```python
from build123d import *

# Parameters (mm, degrees)
BRACKET_SIDE_PROFILE_SKETCH_R        = 3
BRACKET_BODY_EXTRUDE_70MM_DEPTH      = 35
OUTLINE_AND_KEYHOLE_CUT_DEPTH        = 89.24823725
OUTLINE_AND_KEYHOLE_CUT_DEPTH_BACK   = 89.24823725
OUTLINE_AND_KEYHOLE_SKETCH_OUTSIDE_W = 94.54
OUTLINE_AND_KEYHOLE_SKETCH_OUTSIDE_H = 110.471


with BuildPart() as part:
    # Bracket Side Profile Sketch → Bracket Body Extrude 70mm (new, symmetric)
    with BuildSketch(Plane(origin=(0, 0, 0), x_dir=(0, 0, -1), z_dir=(1, 0, 0))):
        with BuildLine():
            Line((1.25, 5.868347297), (1.25, 38))
            ThreePointArc((1.25, 38), (-1.509366946, 51.872274423), (-9.367379182, 63.632620818))
            ThreePointArc((-9.367379182, 63.632620818), (-11.930194847, 69.819805153), (-9.367379182, 76.006989489))
            ThreePointArc((-9.367379182, 76.006989489), (-8.164290412, 77.807539075), (-7.741821818, 79.931432124))
            Line((-7.741821818, 79.931432124), (-10.241821818, 79.931432124))
            ThreePointArc((-10.241821818, 79.931432124), (-10.473989243, 78.764247656), (-11.135146135, 77.774756442))
            ThreePointArc((-11.135146135, 77.774756442), (-14.430194847, 69.819805153), (-11.135146135, 61.864853865))
            ThreePointArc((-11.135146135, 61.864853865), (-3.819065778, 50.915565842), (-1.25, 38))
            Line((-1.25, 38), (-1.25, 5.868347297))
            ThreePointArc((-1.25, 5.868347297), (0, -6), (1.25, 5.868347297))
        make_face()
        Circle(BRACKET_SIDE_PROFILE_SKETCH_R, mode=Mode.SUBTRACT)
    extrude(amount=BRACKET_BODY_EXTRUDE_70MM_DEPTH, both=True)

    # Outline and Keyhole Sketch outside → Outline and Keyhole Cut (cut, two sides: drawn at the far end of the back side and taken through both)
    # profile 1 of 2: a face of its own
    with BuildSketch(Plane.XY.offset(1.25).offset(-OUTLINE_AND_KEYHOLE_CUT_DEPTH_BACK)):
        with Locations((0, 36.9655)):
            Rectangle(OUTLINE_AND_KEYHOLE_SKETCH_OUTSIDE_W, OUTLINE_AND_KEYHOLE_SKETCH_OUTSIDE_H)
        with BuildLine():
            Line((35, -6), (35, 17))
            ThreePointArc((35, 17), (33.314760402, 27.729712921), (28.421329179, 37.426160865))
            ThreePointArc((28.421329179, 37.426160865), (22.418139751, 49.027821234), (20, 61.864853865))
            Line((20, 61.864853865), (20, 79.931432124))
            Line((20, 79.931432124), (-20, 79.931432124))
            Line((-20, 79.931432124), (-20, 61.864853865))
            ThreePointArc((-20, 61.864853865), (-22.418139751, 49.027821234), (-28.421329179, 37.426160865))
            ThreePointArc((-28.421329179, 37.426160865), (-33.314760402, 27.729712921), (-35, 17))
            Line((-35, 17), (-35, -6))
            Line((-35, -6), (-15, -6))
            Line((-15, -6), (-15, 9))
            Line((-15, 9), (15, 9))
            Line((15, 9), (15, -6))
            Line((15, -6), (35, -6))
        make_face(mode=Mode.SUBTRACT)
    # profile 2 of 2: a face of its own
    with BuildSketch(Plane.XY.offset(1.25).offset(-OUTLINE_AND_KEYHOLE_CUT_DEPTH_BACK)):
        with BuildLine():
            Line((7, 49), (7, 39.124143795))
            ThreePointArc((7, 39.124143795), (0, 18.5), (-7, 39.124143795))
            Line((-7, 39.124143795), (-7, 49))
            ThreePointArc((-7, 49), (0, 56), (7, 49))
        make_face()
    extrude(amount=OUTLINE_AND_KEYHOLE_CUT_DEPTH + OUTLINE_AND_KEYHOLE_CUT_DEPTH_BACK, mode=Mode.SUBTRACT)


solid = part.part
```
Input: part model. Units: mm. Frame: model coordinates. A direction names the side the tool comes from. Round coordinates to 2 decimals unless told otherwise and drop trailing zeros. Loops run counter-clockwise (first coordinate to the right, second up) from the corner with the lowest first, then second, coordinate; pieces in that order, holes last. Notation, with made-up numbers: M 47,-24 L 65,-24 A22 cw 65,1 Z; hole C -13.5,5 d10. An arc over 180 degrees is marked long. Answer in a Markdown table with one row per item. Add a question column.
1. Section A-A (y = 0). Output: boundary loops of the cut face in (x, z).
2. Contact query for flat-ended pins moving along their axis: pin 1 (10 mm diameter, centred on x = 17.5, y = 15, fed in from -Z); pin 2 (1 mm diameter, centred on x = 7.5, y = 51.5, fed in from -Z); pin 3 (1.3 mm diameter, centred on y = 43.5, z = 0, fed in from -X); pin 4 (3 mm diameter, centred on x = -26.5, y = 43.5, fed in from +Z). Output: stop coordinate, or through.
3. Mould query, pull axis Z, two halves, no side actions, for faces 1 (the face through (-25, 0, 3)), 2 (the face through (25, -6, 0)), 3 (the face through (0.4, 18.507, -0.008)), 4 (the face through (0.28, 78.78, 10.468)). Classes: released by +Z, released by -Z, zero draft, split by the parting line, or undercut.
4. Section C-C (x = -9.5). Output: boundary loops of the cut face in (y, z).
5. Set-up query: faces 5 (the face through (0, 18, -1.25)), 6 (the face through (0.39, 57.31, 4.32)), 7 (the face through (-20, 71, 13)), 8 (the face through (0, 15, 1.25)). Return all of +Z, -Z, +X, -X, +Y, -Y with unobstructed straight access to the full face (end or side cutting, diameter ignored); none if empty.
6. Section D-D (y = 30). Output: boundary loops of the cut face in (x, z), and give its area (3 significant figures).
7. Section B-B (x = -17). Output: boundary loops of the cut face in (y, z), and give its area (3 significant figures).
8. Ray query, probe 1 along Z at (x, y) = (-25, 0); probe 2 along Z at (x, y) = (-15, 11); probe 3 along Y at (x, z) = (-25, 0). Return the intervals inside material, ascending.
Values follow:
| question | item | result |
|---|---|---|
| 1 | outline | M -35,-6 L -15,-6 L -15,-3 L -35,-3 Z; M -35,3 L -15,3 L -15,6 L -35,6 Z; M 15,-6 L 35,-6 L 35,-3 L 15,-3 Z; M 15,3 L 35,3 L 35,6 L 15,6 Z |
| 2 | pin 1 | z = -1.25 |
| 2 | pin 2 | z = 1.16 |
| 2 | pin 3 | x = -25.08 |
| 2 | pin 4 | through |
| 3 | face 1 | undercut |
| 3 | face 2 | split by the parting line |
| 3 | face 3 | zero draft |
| 3 | face 4 | released by +Z |
| 4 | outline | M 9,-1.25 L 23.52,-1.25 L 23.52,1.25 L 9,1.25 Z; M 36.48,-1.25 L 38,-1.25 A36.25 ccw 63.63,9.37 A8.75 cw 76.01,9.37 A5.55 ccw 79.93,7.74 L 79.93,10.24 A3.05 cw 77.77,11.14 A11.25 ccw 61.86,11.14 A33.75 cw 38,1.25 L 36.48,1.25 Z |
| 5 | face 5 | -Z, +X, -X, +Y |
| 5 | face 6 | -Z, +X, -X |
| 5 | face 7 | +Z, -Z, -X, +Y |
| 5 | face 8 | +Z, +X, -X |
| 6 | outline | M -32.5,-1.25 L -11.5,-1.25 L -11.5,1.25 L -32.5,1.25 Z; M 11.5,-1.25 L 32.5,-1.25 L 32.5,1.25 L 11.5,1.25 Z |
| 6 | area | 105 mm^2 |
| 7 | outline | M 5.87,-1.25 L 38,-1.25 A36.25 ccw 63.63,9.37 A8.75 cw 76.01,9.37 A5.55 ccw 79.93,7.74 L 79.93,10.24 A3.05 cw 77.77,11.14 A11.25 ccw 61.86,11.14 A33.75 cw 38,1.25 L 5.87,1.25 A6 ccw long Z; hole C 0,0 d6 |
| 7 | area | 281 mm^2 |
| 8 | probe 1 | -6 to -3, 3 to 6 |
| 8 | probe 2 | -1.25 to 1.25 |
| 8 | probe 3 | -6 to -3, 3 to 43 |
